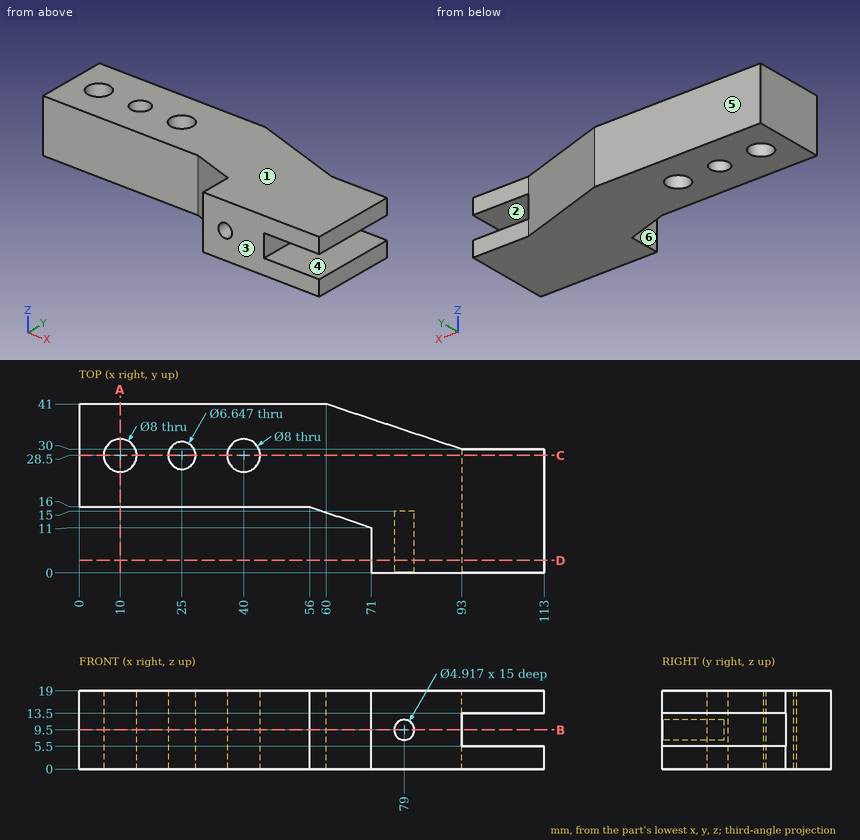
Verification items for this drawing (mm, ordinates from the low corner). A direction names the side the tool comes from. Coordinates: 2 decimals unless noted, no trailing zeros. Order: outer loops, then holes, each group sorted by start corner. A loop starts at its lowest first (then second) coordinate and runs counter-clockwise, first axis right, second up. Notation, with made-up numbers: (15.5, 58) -> (45.5, 58) arc R16 ccw to (45.5, 88) -> close; hole circle Ø1 at (22, -5). An arc over 180 degrees is marked (long way). Put each result on its own line as item: value. Start each with the question number.
1. Cross-section at C-C, the plane y = 28.5. Record the boundary of the cut face in (x, z), then the cut area to 3 significant figures.
2. Cross-section at A-A, the plane x = 10. Record the boundary of the cut face in (y, z).
3. Cross-section at D-D, the plane y = 3. Record the boundary of the cut face in (x, z), then the cut area to 3 significant figures.
4. Access from +Z, -Z, +X, -X, +Y, -Y to the whole of each face (thin tool, end or side, straight path). Record for the marked faces 4, 5 and 6.
5. Cross-section at B-B, the plane z = 9.5. Record the boundary of the cut face in (x, y), then the cut area to 3 significant figures.
6. Material ranges on L1, parallel to Z at x = 79, y = 7.5; L2, parallel to Y at x = 40, z = 14.5; L3, parallel to X at y = 26.5, z = 10, recorded low to high. Write a range as [from, to].
7. Mould release check, pull along Z, two halves, no side actions. Record for the marked faces 1, 2 and 3: released by +Z, released by -Z, zero draft, split by the parting line, or undercut.
8. Go/stop test with flat-tipped pins: pin 1 Ø2.5 at (x, z) = (78, 9) entering from -Y; pin 2 Ø10.5 at (x, y) = (40, 28.5) entering from +Z; pin 3 Ø4.5 at (x, z) = (107, 17) entering from +Y; pin 4 Ø5 at (x, z) = (94.5, 9) entering from +Y. Record where each tip stops, or that it passes through.
Computed:
1. outline: (0, 0) -> (6, 0) -> (6, 19) -> (0, 19) -> close; (14, 0) -> (21.68, 0) -> (21.68, 19) -> (14, 19) -> close; (28.32, 0) -> (36, 0) -> (36, 19) -> (28.32, 19) -> close; (44, 0) -> (113, 0) -> (113, 5.5) -> (93, 5.5) -> (93, 13.5) -> (113, 13.5) -> (113, 19) -> (44, 19) -> close
1. area: 1,560 mm2
2. outline: (16, 0) -> (24.5, 0) -> (24.5, 19) -> (16, 19) -> close; (32.5, 0) -> (41, 0) -> (41, 19) -> (32.5, 19) -> close
3. outline: (71, 0) -> (113, 0) -> (113, 5.5) -> (93, 5.5) -> (93, 13.5) -> (113, 13.5) -> (113, 19) -> (71, 19) -> close; hole circle Ø4.92 at (79, 9.5)
3. area: 619 mm2
4. face 4: +X, +Y, -Y
4. face 5: +Z, -Z, +X, -X, +Y
4. face 6: +Z, -Z, -X, -Y
5. outline: (0, 16) -> (56, 16) -> (71, 11) -> (71, 0) -> (76.54, 0) -> (76.54, 15) -> (81.46, 15) -> (81.46, 0) -> (93, 0) -> (93, 30) -> (60, 41) -> (0, 41) -> close; hole circle Ø8 at (10, 28.5); hole circle Ø6.65 at (25, 28.5); hole circle Ø8 at (40, 28.5)
5. area: 2,320 mm2
6. L1: [0, 7.04], [11.96, 19]
6. L2: [16, 24.5], [32.5, 41]
6. L3: [0, 6.54], [13.46, 22.35], [27.65, 36.54], [43.46, 93]
7. face 1: released by +Z
7. face 2: undercut
7. face 3: zero draft
8. pin 1: y = 15
8. pin 2: z = 19
8. pin 3: y = 30
8. pin 4: y = 30.33
